Input: part model. Units: mm. Frame: model coordinates. A direction names the side the tool comes from. Round coordinates to 2 decimals unless told otherwise and drop trailing zeros. Loops run counter-clockwise (first coordinate to the right, second up) from the corner with the lowest first, then second, coordinate; pieces in that order, holes last. Notation, with made-up numbers: (14, 54.25) -> (65, 54.25) arc R33 ccw to (65, 87.25) -> close; hole circle Ø6 at (74.25, 7). An arc over 180 degrees is marked (long way). One line per question, with ' | ' between items. Start each with the question number.
Q1. Access query for faces 4 (the face through (25, -3, 5)), 5 (the face through (-2.5, 21, 5)), 6 (the face through (27.253, 19.07, 4.879)). Directions: +Z, -Z, +X, -X, +Y, -Y. A direction counts if a zero-diameter tool reaches every point of the face in a straight line with its end or side. Return the directions, or none.
Q2. Cut plane D-D on y = 17. Return loops of the section in (x, z), and give its area (3 significant figures).
Q3. Cut plane A-A on y = -3. Return loops of the section in (x, z).
Q4. Mould query, pull axis X, two halves, no side actions, for faces 1 (the face through (-27.7, 14, 7.1)), 2 (the face through (-32.747, 19.07, 4.879)), 3 (the face through (-22.36, -21.29, 0.25)). Classes: pulls with the +X half, pulls with the -X half, needs draft (parallel to the pull), parting line crosses it, or undercut.
Q5. Cut plane C-C on x = -8. Return loops of the section in (y, z), and give its area (4 significant figures).
Q6. Material intervals for L1, parallel to Z at x = 30, y = 21; L2, parallel to Y at x = -15, z = 8.5; L3, parallel to Y at x = -14.85, z = 4.75, sorted ascending.
Q7. Contact query for flat-ended pins moving along their axis: P1, Ø4.5, axis at y = -4.5, z = 3, coming from the -X side; P2, Ø1.5, axis at y = 7.5, z = 2.5, coming from the +X side; P3, Ø2.5, axis at x = -0.5, z = 4, coming from the +Y side. Output: stop coordinate, or through.
Q8. Cut plane B-B on z = 5. State how many separate pieces and enclosed holes the cut face has, and give its area (3 significant figures).
from build123d import *

# Parameters (mm, degrees)
SKETCH_1_W              = 70
SKETCH_1_H              = 48
EXTRUDE_1_DEPTH         = 10
SKETCH_2_W              = 10
SKETCH_2_H              = 38
CUT_EXTRUDE_1_DEPTH     = 44.600458713
SKETCH_3_R              = 17
CUT_EXTRUDE_2_DEPTH     = 44.600458713
HOLE_WIZARD_M4_2_D      = 3.3
HOLE_WIZARD_5_5_5_5_1_D = 5.5
CHAMFER_1_SIZE          = 5
SKETCH_12_W             = 5
SKETCH_12_H             = 5
CUT_EXTRUDE_3_DEPTH     = 44.600458713
CHAMFER_2_SIZE          = 0.5


with BuildPart() as part:
    # 草图1 → 凸台-拉伸1 (new body)
    with BuildSketch(Plane.XY):
        Rectangle(SKETCH_1_W, SKETCH_1_H)
    extrude(amount=EXTRUDE_1_DEPTH)

    # 草图2 → 切除-拉伸1 (cut, through all)
    with BuildSketch(Plane.XY.offset(10)):
        with Locations((-30, -5)):
            Rectangle(SKETCH_2_W, SKETCH_2_H)
        with Locations((30, -5)):
            Rectangle(SKETCH_2_W, SKETCH_2_H)
    extrude(amount=-CUT_EXTRUDE_1_DEPTH, mode=Mode.SUBTRACT)

    # 草图3 → 切除-拉伸2 (cut, through all)
    with BuildSketch(Plane(origin=(0, 0, 0), x_dir=(-1, 0, 0), z_dir=(0, 0, -1))):
        with Locations((0, -3)):
            Circle(SKETCH_3_R)
    extrude(amount=-CUT_EXTRUDE_2_DEPTH, mode=Mode.SUBTRACT)

    # M4 螺纹孔2 (through all)
    with Locations(Plane.XY.offset(10)):
        with Locations((14.85, -17.85), (-14.85, -17.85), (-14.85, 11.85), (14.85, 11.85)):
            Hole(HOLE_WIZARD_M4_2_D / 2)

    # Ø5.5 (5.5) 直径孔1 (through all)
    with Locations(Plane(origin=(0, 14, 0), x_dir=(-1, 0, 0), z_dir=(0, -1, 0))):
        with Locations((-30, -5), (30, -5)):
            Hole(HOLE_WIZARD_5_5_5_5_1_D / 2)

    # 倒角1
    chamfer_1_edges = [part.edges().sort_by_distance(p)[0] for p in [
        (-25, -24, 5),
        (25, -24, 5),
    ]]
    chamfer(chamfer_1_edges, length=CHAMFER_1_SIZE)

    # 草图12 → 切除-拉伸3 (cut, through all)
    with BuildSketch(Plane.XY.offset(10)):
        with Locations((0, 21.5)):
            Rectangle(SKETCH_12_W, SKETCH_12_H)
    extrude(amount=-CUT_EXTRUDE_3_DEPTH, mode=Mode.SUBTRACT)

    # 倒角2
    chamfer_2_edges = [part.edges().sort_by_distance(p)[0] for p in [
        (-35, 19, 10),
        (-30, 14, 0),
        (-35, 14, 5),
        (-30, 14, 10),
        (35, 19, 0),
        (35, 19, 10),
        (25, -2.5, 0),
        (30, 14, 0),
        (35, 14, 5),
        (30, 14, 10),
        (25, -2.5, 10),
        (-35, 19, 0),
        (18.75, 24, 0),
        (18.75, 24, 10),
        (-35, 24, 5),
        (35, 24, 5),
        (-25, -2.5, 10),
        (-25, -2.5, 0),
        (0, -24, 10),
        (22.5, -21.5, 10),
        (-22.5, -21.5, 10),
        (0, -24, 0),
        (22.5, -21.5, 0),
        (-22.5, -21.5, 0),
        (-18.75, 24, 0),
        (-18.75, 24, 10),
        (-2.5, 21.5, 0),
        (2.5, 21.5, 0),
        (0, 19, 0),
        (-2.5, 21.5, 10),
        (0, 19, 10),
        (2.5, 21.5, 10),
    ]]
    chamfer(chamfer_2_edges, length=CHAMFER_2_SIZE)


solid = part.part
Results:
1) face 4: +Z, -Z, +X, -Y | face 5: +Z, -Z, +Y | face 6: +Y, -Y
2) outline: (-35, 0.5) -> (-34.5, 0) -> (34.5, 0) -> (35, 0.5) -> (35, 9.5) -> (34.5, 10) -> (-34.5, 10) -> (-35, 9.5) -> close; hole circle Ø5.5 at (-30, 5); hole circle Ø5.5 at (30, 5) | area: 652 mm^2
3) outline: (-25, 0.5) -> (-24.5, 0) -> (-17, 0) -> (-17, 10) -> (-24.5, 10) -> (-25, 9.5) -> close; (17, 0) -> (24.5, 0) -> (25, 0.5) -> (25, 9.5) -> (24.5, 10) -> (17, 10) -> close
4) face 1: needs draft | face 2: undercut | face 3: pulls with the -X half
5) outline: (-24, 0.5) -> (-23.5, 0) -> (-18, 0) -> (-18, 10) -> (-23.5, 10) -> (-24, 9.5) -> close; (12, 0) -> (23.5, 0) -> (24, 0.5) -> (24, 9.5) -> (23.5, 10) -> (12, 10) -> close | area: 179.5 mm^2
6) L1: 0 to 2.25, 7.75 to 10 | L2: -24 to -19.49, -16.21 to -11, 5 to 10.21, 13.49 to 24 | L3: -24 to -19.5, -16.2 to -11.28, 5.28 to 10.2, 13.5 to 24
7) P1: x = -25 | P2: x = 25 | P3: y = 19
8) separate pieces: 3 | enclosed holes: 5 | area: 1,500 mm^2
